Source: CAD feature listing. Evaluate the final solid. Frame: model axes, mm. A direction names the side the tool comes from. Give positions to 0.01 mm unless a question says otherwise; leave off trailing zeros. Write each loop counter-clockwise with the first axis right and the second up, starting at its lowest first coordinate (ties: lowest second). Pieces come first, ordered by that corner, then holes.
```python
from build123d import *


with BuildPart() as part:
    # Sketch1 → Revolve1 (revolve)
    with BuildSketch(Plane.XY, mode=Mode.PRIVATE) as revolve1_sk:
        Polygon((1.1, 0), (2.9, 0), (3, 0.1), (3, 19), (2.5, 19), (2.5, 21), (3, 21), (3, 26.9), (2.9, 27), (1.6, 27), (1.498148466, 26.900017142), (1.001851534, 0.099982858), align=None)
    revolve(revolve1_sk.sketch.rotate(Axis((0, 0, 0), (0, 1, 0)), 90), axis=Axis((0, 0, 0), (0, 1, 0)))


solid = part.part
```
1. Line query: probe 1 along Y at (x, z) = (-2.4, -0.85); probe 2 along Z at (x, y) = (-2.6, 24.5); probe 3 along X at (y, z) = (8, -0.6). Output: solid intervals per line, ascending.
2. Section query B-B (y = 13.75). Return loops of the section in (x, z).
3. Section query A-A (y = 23). Return loops of the section in (x, z).
4. Pin query (flat end, axial travel): P1, Ø1.8, axis at x = -0.5, z = 0, coming from the -Y side; P2, Ø2, axis at x = -1.5, y = 15, coming from the +Z side. Return the tip coordinate at first contact, or that it passes through.
5. Access query for faces 5 (the flat face through (-0.04, 0, 1.25)), 6 (the flat face through (-2, 19, 2)), 7 (the conical face through (1.106, 13.312, -0.575)). Directions: +Z, -Z, +X, -X, +Y, -Y. A direction counts if a zero-diameter tool reaches every point of the face in a straight line with its end or side. Return the directions, or none.
6. Pull-direction query (Y, two-part tool) for faces 1 (the flat face through (1.25, 27, -1.25)), 2 (the cylindrical face through (-0.1, 20, 2.5)), 3 (the flat face through (-2, 21, -2)), 4 (the cylindrical face through (-0.9, 23.99, -2.86)); classes: pulls with the +Y half, pulls with the -Y half, needs draft (parallel to the pull), parting line crosses it, or undercut.
The answers:
1. probe 1: y = 0 to 19, 21 to 27
1. probe 2: z = -1.5 to 1.5
1. probe 3: x = -2.94 to -0.98, 0.98 to 2.94
2. outline: circle Ø6 at (0, 0); hole circle Ø2.51 at (0, 0)
3. outline: circle Ø6 at (0, 0); hole circle Ø2.85 at (0, 0)
4. P1: stops at y = 0
4. P2: stops at z = 2.96
5. face 5: +Z, -Z, +X, -X, -Y
5. face 6: none
5. face 7: +Y
6. face 1: pulls with the +Y half
6. face 2: undercut
6. face 3: undercut
6. face 4: needs draft
